from build123d import *
from OCP.BRepFilletAPI import BRepFilletAPI_MakeChamfer

# Parameters (mm, degrees)
SKETCH1_W           = 10
SKETCH1_H           = 35
BOSS_EXTRUDE1_DEPTH = 15
CHAMFER1_SIZE       = 8
CHAMFER1_SIZE2      = 5
BOSS_EXTRUDE2_DEPTH = 35
CHAMFER2_SIZE       = 2
CHAMFER3_SIZE       = 1
CHAMFER3_SIZE2      = 1.414213562


with BuildPart() as part:
    # Sketch1 → Revolve1 (revolve)
    with BuildSketch(Plane(origin=(0, 0, 0), x_dir=(1, 0, 0), z_dir=(0, 1, 0)), mode=Mode.PRIVATE) as revolve1_sk:
        with Locations((35, 17.5)):
            Rectangle(SKETCH1_W, SKETCH1_H)
        Polygon((0, 0), (30, 0), (30, 35), (0, 26.961524227), align=None)
    revolve(revolve1_sk.sketch.rotate(Axis((0, 0, 0), (1, 0, 0)), 180), axis=Axis((0, 0, 0), (1, 0, 0)))

    # Sketch2 → Boss-Extrude1 (add)
    with BuildSketch(Plane(origin=(40, 0, 0), x_dir=(0, 0, -1), z_dir=(1, 0, 0))):
        with BuildLine():
            Line((-44, -60), (44, -60))
            ThreePointArc((44, -60), (55.313708499, -55.313708499), (60, -44))
            Line((60, -44), (60, 44))
            ThreePointArc((60, 44), (55.313708499, 55.313708499), (44, 60))
            Line((44, 60), (-44, 60))
            ThreePointArc((-44, 60), (-55.313708499, 55.313708499), (-60, 44))
            Line((-60, 44), (-60, -44))
            ThreePointArc((-60, -44), (-55.313708499, -55.313708499), (-44, -60))
        make_face()
    extrude(amount=BOSS_EXTRUDE1_DEPTH)

    # Chamfer1: one chamfer whose edges measure the first distance from different faces: ONE call of the kernel's chamfer builder (chamfer() names one face for all edges)
    chamfer1_edges_1 = [part.edges().sort_by_distance(p)[0] for p in [
        (55, -55.313708499, 55.313708499),
    ]]
    chamfer1_side_1 = [part.faces().sort_by_distance(p)[0] for p in [
        (47.5, -55.313708499, 55.313708499),
    ]]
    chamfer1_edges_2 = [part.edges().sort_by_distance(p)[0] for p in [
        (55, -60, 0),
    ]]
    chamfer1_side_2 = [part.faces().sort_by_distance(p)[0] for p in [
        (47.5, -60, 0),
    ]]
    chamfer1_edges_3 = [part.edges().sort_by_distance(p)[0] for p in [
        (55, -55.313708499, -55.313708499),
    ]]
    chamfer1_side_3 = [part.faces().sort_by_distance(p)[0] for p in [
        (47.5, -55.313708499, -55.313708499),
    ]]
    chamfer1_edges_4 = [part.edges().sort_by_distance(p)[0] for p in [
        (55, 0, -60),
    ]]
    chamfer1_side_4 = [part.faces().sort_by_distance(p)[0] for p in [
        (47.5, 0, -60),
    ]]
    chamfer1_edges_5 = [part.edges().sort_by_distance(p)[0] for p in [
        (55, 55.313708499, -55.313708499),
    ]]
    chamfer1_side_5 = [part.faces().sort_by_distance(p)[0] for p in [
        (47.5, 55.313708499, -55.313708499),
    ]]
    chamfer1_edges_6 = [part.edges().sort_by_distance(p)[0] for p in [
        (55, 60, 0),
    ]]
    chamfer1_side_6 = [part.faces().sort_by_distance(p)[0] for p in [
        (47.5, 60, 0),
    ]]
    chamfer1_edges_7 = [part.edges().sort_by_distance(p)[0] for p in [
        (55, 55.313708499, 55.313708499),
    ]]
    chamfer1_side_7 = [part.faces().sort_by_distance(p)[0] for p in [
        (47.5, 55.313708499, 55.313708499),
    ]]
    chamfer1_edges_8 = [part.edges().sort_by_distance(p)[0] for p in [
        (55, 0, 60),
    ]]
    chamfer1_side_8 = [part.faces().sort_by_distance(p)[0] for p in [
        (47.5, 0, 60),
    ]]
    chamfer1 = BRepFilletAPI_MakeChamfer(part.part.solid().wrapped)
    for e in chamfer1_edges_1:
        chamfer1.Add(CHAMFER1_SIZE, CHAMFER1_SIZE2, e.wrapped, chamfer1_side_1[0].wrapped)  # the first distance lies on this face
    for e in chamfer1_edges_2:
        chamfer1.Add(CHAMFER1_SIZE, CHAMFER1_SIZE2, e.wrapped, chamfer1_side_2[0].wrapped)  # the first distance lies on this face
    for e in chamfer1_edges_3:
        chamfer1.Add(CHAMFER1_SIZE, CHAMFER1_SIZE2, e.wrapped, chamfer1_side_3[0].wrapped)  # the first distance lies on this face
    for e in chamfer1_edges_4:
        chamfer1.Add(CHAMFER1_SIZE, CHAMFER1_SIZE2, e.wrapped, chamfer1_side_4[0].wrapped)  # the first distance lies on this face
    for e in chamfer1_edges_5:
        chamfer1.Add(CHAMFER1_SIZE, CHAMFER1_SIZE2, e.wrapped, chamfer1_side_5[0].wrapped)  # the first distance lies on this face
    for e in chamfer1_edges_6:
        chamfer1.Add(CHAMFER1_SIZE, CHAMFER1_SIZE2, e.wrapped, chamfer1_side_6[0].wrapped)  # the first distance lies on this face
    for e in chamfer1_edges_7:
        chamfer1.Add(CHAMFER1_SIZE, CHAMFER1_SIZE2, e.wrapped, chamfer1_side_7[0].wrapped)  # the first distance lies on this face
    for e in chamfer1_edges_8:
        chamfer1.Add(CHAMFER1_SIZE, CHAMFER1_SIZE2, e.wrapped, chamfer1_side_8[0].wrapped)  # the first distance lies on this face
    add(Compound.cast(chamfer1.Shape()), mode=Mode.REPLACE)

    # Sketch3 → Boss-Extrude2 (add)
    with BuildSketch(Plane(origin=(55, 0, 0), x_dir=(0, 0, -1), z_dir=(1, 0, 0))):
        with BuildLine():
            Line((-44.591144521, -54), (44.591144521, -54))
            ThreePointArc((44.591144521, -54), (51.244210033, -51.244210033), (54, -44.591144521))
            Line((54, -44.591144521), (54, 44.591144521))
            ThreePointArc((54, 44.591144521), (51.244210033, 51.244210033), (44.591144521, 54))
            Line((44.591144521, 54), (-44.591144521, 54))
            ThreePointArc((-44.591144521, 54), (-51.244210033, 51.244210033), (-54, 44.591144521))
            Line((-54, 44.591144521), (-54, -44.591144521))
            ThreePointArc((-54, -44.591144521), (-51.244210033, -51.244210033), (-44.591144521, -54))
        make_face()
    extrude(amount=BOSS_EXTRUDE2_DEPTH)

    # Chamfer2
    chamfer2_edges = [part.edges().sort_by_distance(p)[0] for p in [
        (90, 51.244210033, -51.244210033),
        (90, 54, 0),
        (90, 51.244210033, 51.244210033),
        (90, 0, 54),
        (90, -51.244210033, 51.244210033),
        (90, -54, 0),
        (90, -51.244210033, -51.244210033),
        (90, 0, -54),
    ]]
    chamfer(chamfer2_edges, length=CHAMFER2_SIZE)

    # Chamfer3
    chamfer3_edges = [part.edges().sort_by_distance(p)[0] for p in [
        (0, 0, -26.961524227),
    ]]
    chamfer3_side = [part.faces().sort_by_distance(p)[0] for p in [
        (15, 0, -30.980762114),
    ]]
    chamfer(chamfer3_edges, length=CHAMFER3_SIZE, length2=CHAMFER3_SIZE2, reference=chamfer3_side[0])


solid = part.part
Check sheet for the modelled part. Datum: model origin and axes. Units: mm. A direction names the side the tool comes from. Round coordinates to 2 decimals unless told otherwise and drop trailing zeros. Loops run counter-clockwise (first coordinate to the right, second up) from the corner with the lowest first, then second, coordinate; pieces in that order, holes last. Notation, with made-up numbers: M 74,-40 L 112,-40 A24 ccw 112,-23 Z; hole C 7.25,33.25 d10. An arc over 180 degrees is marked long. One line per question, with ' | ' between items. Start each with the question number.
Item 1: Gauge pin test, flat ends, axial feed: pin 1 Ø3 at (y, z) = (-24.5, -28.5) entering from -X; pin 2 Ø12 at (x, z) = (69.5, -20) entering from +Y; pin 3 Ø4 at (x, y) = (39.5, 7.5) entering from +Z; pin 4 Ø2 at (x, z) = (54, 30) entering from +Y. Record the tip position at first contact, or that the pin passes through.
Item 2: Scan lines: probe 1 along Y at (x, z) = (63, -29); probe 2 along X at (y, z) = (-9, -46.5). Record each from-to range of solid material in increasing order.
Item 3: Section check D-D (z = 39). Record the boundary of the cut face in (x, y), and give its area (3 significant figures).
Item 4: Section check A-A (x = 82.5). Record the boundary of the cut face in (y, z), and give its area (3 significant figures).
Item 5: Set-up check for faces 1 (the face through (40, 28, 28)), 2 (the face through (71.27, -51.32, -51.17)), 3 (the face through (71.27, 51.17, -51.32)), 4 (the face through (71.27, 51.32, 51.17)): record each of +Z, -Z, +X, -X, +Y, -Y from which the full face is reachable in a straight line by a thin tool's end or side.
Item 6: Section check B-B (z = 0). Record the boundary of the cut face in (x, y), and give its area (3 significant figures).
Worked out:
1) pin 1: x = 40 | pin 2: y = 54 | pin 3: z = 60 | pin 4: y = 56.25
2) probe 1: -54 to 54 | probe 2: 40 to 90
3) outline: M 40,-60 L 47,-60 L 55,-55 L 55,-54 L 88,-54 L 90,-52 L 90,52 L 88,54 L 55,54 L 55,55 L 47,60 L 40,60 Z | area: 5,540 mm^2
4) outline: M -54,-44.59 A9.41 ccw -44.59,-54 L 44.59,-54 A9.41 ccw 54,-44.59 L 54,44.59 A9.41 ccw 44.59,54 L -44.59,54 A9.41 ccw -54,44.59 Z | area: 11,600 mm^2
5) face 1: -X | face 2: -Z, +X, -Y | face 3: -Z, +X, +Y | face 4: +Z, +X, +Y
6) outline: M 0,-25.55 L 0.97,-27.22 L 30,-35 L 40,-35 L 40,-60 L 47,-60 L 55,-55 L 55,-54 L 88,-54 L 90,-52 L 90,52 L 88,54 L 55,54 L 55,55 L 47,60 L 40,60 L 40,35 L 30,35 L 0.97,27.22 L 0,25.55 Z | area: 8,090 mm^2
